The model under review builds one solid part; all positions refer to its coordinate system, in mm. A direction names the side the tool comes from. Round coordinates to 2 decimals unless told otherwise and drop trailing zeros. Write each loop counter-clockwise with the first axis right and the second up, starting at its lowest first coordinate (ties: lowest second). Pieces come first, ordered by that corner, then holes. Notation, with made-up numbers: (-7, 89) -> (52, 89) arc R18 cw to (52, 105) -> close; hole circle Ø7 at (14.5, -21.5). An arc over 180 degrees is marked (long way). Return JSON: item names as keys, results as strings. Group by question number.
1. Take a section at B-B, the plane z = 36. Write out the cut boundary in (x, y), then the cut area to 4 significant figures.
2. Clearance check with flat-ended pins moving along their axes: P1, Ø1.5, axis at x = 28, z = 6.5, coming from the -Y side; P2, Ø8, axis at x = 46.5, z = 38.5, coming from the +Y side; P3, Ø10, axis at y = 36.5, z = 39, coming from the +X side; P4, Ø9, axis at x = 20, y = 25, coming from the -Z side. State where each tip first meets the part, or that it passes through.
3. Take a section at D-D, the plane y = 11. Write out the cut boundary in (x, z).
4. Take a section at A-A, the plane x = 20. Write out the cut boundary in (y, z).
5. For line 1 along X through (y, z) = (11.5, 35); line 2 along X through (y, z) = (25.5, 36); line 3 along Z through (x, y) = (12, 18), list the stretches that pass through material, from the lowest coordinate up. Write a range as from..to.
6. Tool access review of faces 1 (the flat face through (40, 32, 10)), 2 (the flat face through (13, 31, 40)), 3 (the flat face through (55, 29, 30)): name each direction out of +Z, -Z, +X, -X, +Y, -Y from which nothing blocks a thin tool from reaching the whole face with its end or side.
7. Take a section at C-C, the plane z = 43. Write out the cut boundary in (x, y), then the cut area to 3 significant figures.
8. Mouldability with a two-part tool opening along X and no side actions: class faces 4 (the cylindrical face through (14.5, 30.1, 45.1)), 5 (the cylindrical face through (14.5, 19.9, 5.1)), 6 (the flat face through (36, 20, 0)), 7 (the flat face through (40, 32, 40)) as pulls with the +X half, pulls with the -X half, needs draft (parallel to the pull), parting line crosses it, or undercut.
from build123d import *

# Parameters (mm, degrees)
BRACKET_BASE_50MM_DEPTH    = 50
HOLE_1_SKETCH_R            = 7.5
HOLE_1_CUT_10MM_DEEP_DEPTH = 10
HOLE_START                 = -10
HOLE_2_SKETCH_R            = 7.5
HOLE_2_CUT_10MM_DEEP_DEPTH = 10
RAISED_BOSS_SKETCH_W       = 10
RAISED_BOSS_SKETCH_H       = 10
RAISED_BOSS_35MM_DEPTH     = 35
GUSSET_RIB_10MM_REACH      = 112.227
GUSSET_RIB_SKETCH_WALL_W   = 279.462848106
GUSSET_RIB_SKETCH_WALL_H   = 10
SQUARE_POCKET_SKETCH_W     = 20
SQUARE_POCKET_SKETCH_H     = 30
SQUARE_POCKET_CUT_DEPTH    = 119.427192823


with BuildPart() as part:
    # Bracket Profile Sketch → Bracket Base 50mm (new body)
    with BuildSketch(Plane.XY):
        Polygon((0, 0), (95, 0), (95, 15), (40, 15), (40, 50), (0, 50), align=None)
    extrude(amount=BRACKET_BASE_50MM_DEPTH)

    # Hole 1 Sketch → Hole 1 Cut 10mm Deep (cut)
    with BuildSketch(Plane.XY.offset(50)):
        with Locations((20, 25)):
            Circle(HOLE_1_SKETCH_R)
    extrude(amount=-HOLE_1_CUT_10MM_DEEP_DEPTH, mode=Mode.SUBTRACT)

    # Hole 2 Sketch → Hole 2 Cut 10mm Deep (cut)
    with BuildSketch(Plane(origin=(0, 0, 0), x_dir=(-1, 0, 0), z_dir=(0, 0, -1)).offset(HOLE_START)):
        with Locations(Location((-20, 25, 0), (0, 0, 180))):
            Circle(HOLE_2_SKETCH_R)
    extrude(amount=HOLE_2_CUT_10MM_DEEP_DEPTH, mode=Mode.SUBTRACT)

    # Raised Boss Sketch → Raised Boss 35mm (add)
    with BuildSketch(Plane(origin=(0, 50, 0), x_dir=(1, 0, 0), z_dir=(0, 1, 0))):
        with Locations((45, -25)):
            Rectangle(RAISED_BOSS_SKETCH_W, RAISED_BOSS_SKETCH_H)
    extrude(amount=-RAISED_BOSS_35MM_DEPTH)

    # Gusset Rib Sketch wall → Gusset Rib 10mm (add, up to next)
    with BuildSketch(Plane(origin=(72.5, 32.5, 25), x_dir=(0.789352217376, -0.613940613515, 0), z_dir=(0.613940613515, 0.789352217376, 0)), mode=Mode.PRIVATE) as gusset_rib_10mm_sk1:
        Rectangle(GUSSET_RIB_SKETCH_WALL_W, GUSSET_RIB_SKETCH_WALL_H)
    gusset_rib_10mm_tool1 = extrude(gusset_rib_10mm_sk1.sketch, amount=-GUSSET_RIB_10MM_REACH, mode=Mode.PRIVATE) - part.part
    add(gusset_rib_10mm_tool1.solids().sort_by_distance((72.5, 32.5, 25))[0])

    # Square Pocket Sketch → Square Pocket Cut (cut, through all)
    with BuildSketch(Plane(origin=(0, 50, 0), x_dir=(1, 0, 0), z_dir=(0, 1, 0))):
        with Locations((20, -25)):
            Rectangle(SQUARE_POCKET_SKETCH_W, SQUARE_POCKET_SKETCH_H)
    extrude(amount=-SQUARE_POCKET_CUT_DEPTH, mode=Mode.SUBTRACT)


solid = part.part
Output:
{
 "1": {"outline": "(0, 0) -> (10, 0) -> (10, 50) -> (0, 50) -> close; (30, 0) -> (95, 0) -> (95, 15) -> (40, 15) -> (40, 50) -> (30, 50) -> close", "area": "1,825 mm^2"},
 "2": {"P1": "stops at y = 0", "P2": "stops at y = 15", "P3": "stops at x = 40", "P4": "passes through"},
 "3": {"outline": "(0, 0) -> (95, 0) -> (95, 50) -> (0, 50) -> close; hole (10, 10) -> (30, 10) -> (30, 40) -> (10, 40) -> close"},
 "4": {"outline": "(0, 0) -> (17.5, 0) -> (17.5, 10) -> (0, 10) -> close; (0, 40) -> (17.5, 40) -> (17.5, 50) -> (0, 50) -> close; (32.5, 0) -> (50, 0) -> (50, 10) -> (32.5, 10) -> close; (32.5, 40) -> (50, 40) -> (50, 50) -> (32.5, 50) -> close"},
 "5": {"line 1": "x = 0..10, 30..95", "line 2": "x = 0..10, 30..40", "line 3": "z = 0..10, 40..50"},
 "6": {"face 1": "-Z, +X, +Y", "face 2": "+Y, -Y", "face 3": "+Z, +X, +Y"},
 "7": {"outline": "(0, 0) -> (95, 0) -> (95, 15) -> (40, 15) -> (40, 50) -> (0, 50) -> close; hole circle Ø15 at (20, 25)", "area": "2,650 mm^2"},
 "8": {"face 4": "undercut", "face 5": "undercut", "face 6": "needs draft", "face 7": "pulls with the +X half"}
}
